```python
from build123d import *

# Parameters (mm, degrees)
SKETCH1_W           = 130
SKETCH1_H           = 40
BOSS_EXTRUDE1_DEPTH = 10
BOSS_EXTRUDE2_DEPTH = 30
SKETCH3_W           = 110
SKETCH3_H           = 10
CUT_EXTRUDE1_DEPTH  = 40
SKETCH4_R           = 7.5
CUT_EXTRUDE2_DEPTH  = 40
SKETCH5_R           = 14
CUT_EXTRUDE3_DEPTH  = 40
SKETCH6_R           = 12.5
CUT_EXTRUDE4_DEPTH  = 10


with BuildPart() as part:
    # Sketch1 → Boss-Extrude1 (new body)
    with BuildSketch(Plane.XY):
        Rectangle(SKETCH1_W, SKETCH1_H)
    extrude(amount=BOSS_EXTRUDE1_DEPTH)

    # Sketch2 → Boss-Extrude2 (add)
    with BuildSketch(Plane.XY.offset(10)):
        Polygon((-65, 20), (55, 20), (73, 5), (73, -5), (55, -20), (-65, -20), align=None)
    extrude(amount=BOSS_EXTRUDE2_DEPTH)

    # Sketch3 → Cut-Extrude1 (cut)
    with BuildSketch(Plane.XZ.offset(20)):
        with Locations((-10, 35)):
            Rectangle(SKETCH3_W, SKETCH3_H)
    extrude(amount=-CUT_EXTRUDE1_DEPTH, mode=Mode.SUBTRACT)

    # Sketch4 → Cut-Extrude2 (cut)
    with BuildSketch(Plane(origin=(0, 0, 0), x_dir=(-1, 0, 0), z_dir=(0, 0, -1))):
        with Locations((-35, 0)):
            Circle(SKETCH4_R)
        with Locations((35, 0)):
            Circle(SKETCH4_R)
    extrude(amount=-CUT_EXTRUDE2_DEPTH, mode=Mode.SUBTRACT)

    # Sketch5 → Cut-Extrude3 (cut)
    with BuildSketch(Plane.XY.offset(30)):
        with Locations((-35, 0)):
            Circle(SKETCH5_R)
        with Locations((35, 0)):
            Circle(SKETCH5_R)
    extrude(amount=CUT_EXTRUDE3_DEPTH, mode=Mode.SUBTRACT)

    # Sketch6 → Cut-Extrude4 (cut)
    with BuildSketch(Plane.XY.offset(30)):
        with Locations((35, 0)):
            Circle(SKETCH6_R)
        with Locations((-35, 0)):
            Circle(SKETCH6_R)
    extrude(amount=-CUT_EXTRUDE4_DEPTH, mode=Mode.SUBTRACT)


solid = part.part
```
Check sheet for the modelled part. Datum: model origin and axes. Units: mm. A direction names the side the tool comes from. Round coordinates to 2 decimals unless told otherwise and drop trailing zeros. Loops run counter-clockwise (first coordinate to the right, second up) from the corner with the lowest first, then second, coordinate; pieces in that order, holes last. Notation, with made-up numbers: (31, 25.5) -> (66, 25.5) arc R32 ccw to (66, 54.5) -> close; hole circle Ø10 at (39.5, 27.5). An arc over 180 degrees is marked (long way). Answer in a Markdown table with one row per item.
Q1. Go/stop test with flat-tipped pins: P1, Ø7.5, axis at x = -38.5, y = 2.5, coming from the +Z side; P2, Ø20, axis at x = -30, y = 1.5, coming from the +Z side; P3, Ø5, axis at y = -14, z = 35.5, coming from the -X side; P4, Ø7.5, axis at x = 34, y = -2, coming from the +Z side. Record where each tip stops, or that it passes through.
Data:
| item | result |
|---|---|
| P1 | stops at z = 20 |
| P2 | stops at z = 30 |
| P3 | stops at x = 45 |
| P4 | passes through |
Q2. Release check for a two-part mould opening along X. For faces 1 (the face through (42.493, 0.33, 9.86)), 2 (the face through (62, -18, 10)), 3 (the face through (-65, 0, 15)) record: released by +X, released by -X, zero draft, split by the parting line, or undercut.
Data:
| item | result |
|---|---|
| face 1 | undercut |
| face 2 | zero draft |
| face 3 | released by -X |
Q3. Sectioned sample at B-B on x = -35. Enter the section's corners in (y, z).
Data:
| item | result |
|---|---|
| outline | (-20, 0) -> (-7.5, 0) -> (-7.5, 20) -> (-12.5, 20) -> (-12.5, 30) -> (-20, 30) -> close; (7.5, 0) -> (20, 0) -> (20, 30) -> (12.5, 30) -> (12.5, 20) -> (7.5, 20) -> close |
Q4. Thickness scan on L1, parallel to Y at x = -35, z = 8; L2, parallel to Y at x = 35, z = 25.25; L3, parallel to X at y = -11, z = 24. Record the ranges inside material, lowest first.
Data:
| item | result |
|---|---|
| L1 | y = -20 to -7.5, 7.5 to 20 |
| L2 | y = -20 to -12.5, 12.5 to 20 |
| L3 | x = -65 to -40.94, -29.06 to 29.06, 40.94 to 65.8 |
Q5. Sectioned sample at D-D on z = 34.5. Enter the section's corners in (x, y), then the cut area to 3 significant figures.
Data:
| item | result |
|---|---|
| outline | (45, -20) -> (55, -20) -> (73, -5) -> (73, 5) -> (55, 20) -> (45, 20) -> (45, 9.8) arc R14 cw to (45, -9.8) -> close |
| area | 796 mm^2 |
Q6. Sectioned sample at A-A on y = 0. Enter the section's corners in (x, z), then the cut area to 3 significant figures.
Data:
| item | result |
|---|---|
| outline | (-65, 0) -> (-42.5, 0) -> (-42.5, 20) -> (-47.5, 20) -> (-47.5, 30) -> (-65, 30) -> close; (-27.5, 0) -> (27.5, 0) -> (27.5, 20) -> (22.5, 20) -> (22.5, 30) -> (-22.5, 30) -> (-22.5, 20) -> (-27.5, 20) -> close; (42.5, 0) -> (65, 0) -> (65, 10) -> (73, 10) -> (73, 40) -> (49, 40) -> (49, 30) -> (47.5, 30) -> (47.5, 20) -> (42.5, 20) -> close |
| area | 3,200 mm^2 |
Q7. Set-up check for faces 4 (the face through (64.126, -12.395, 24.79)), 5 (the face through (22.512, 0.55, 25.07)), 6 (the face through (62, 18, 10)): record each of +Z, -Z, +X, -X, +Y, -Y from which the full face is reachable in a straight line by a thin tool's end or side.
Data:
| item | result |
|---|---|
| face 4 | +Z, +X, -Y |
| face 5 | +Z |
| face 6 | +Z, +X, +Y |
Q8. Sectioned sample at C-C on z = 3. Enter the section's corners in (x, y), then the cut area to 3 significant figures.
Data:
| item | result |
|---|---|
| outline | (-65, -20) -> (65, -20) -> (65, 20) -> (-65, 20) -> close; hole circle Ø15 at (-35, 0); hole circle Ø15 at (35, 0) |
| area | 4,850 mm^2 |
